Read the model definition and answer for the solid it produces. Units are mm, in the model's axes. A direction names the side the tool comes from. Give positions to 0.01 mm unless a question says otherwise; leave off trailing zeros. Order: outer loops, then holes, each group sorted by start corner. A loop starts at its lowest first (then second) coordinate and runs counter-clockwise, first axis right, second up. Notation, with made-up numbers: M 23,86 L 42,86 A25 ccw 42,123 Z; hole C 61,73.25 d2. An arc over 180 degrees is marked long. One line per item, written item: value.
from build123d import *
from OCP.BRepFilletAPI import BRepFilletAPI_MakeChamfer

# Parameters (mm, degrees)
SKETCH2_R           = 110
BOSS_EXTRUDE1_DEPTH = 26
CUT_EXTRUDE1_DEPTH  = 26
CHAMFER1_SIZE       = 2
CHAMFER2_SIZE       = 10
CHAMFER2_SIZE2      = 5.773502692
SKETCH4_R           = 85
CUT_EXTRUDE2_DEPTH  = 26
CHAMFER3_SIZE       = 2


with BuildPart() as part:
    # Sketch2 → Boss-Extrude1 (new body)
    with BuildSketch(Plane.XY):
        with Locations(Location((0, 0, 0), (0, 0, 180))):
            Circle(SKETCH2_R)
    extrude(amount=BOSS_EXTRUDE1_DEPTH)

    # Sketch3 → Cut-Extrude1 (cut)
    with BuildSketch(Plane.XY.offset(26)):
        with BuildLine():
            Line((-8, 109.954040528), (-8, 103))
            Line((-8, 103), (8, 103))
            Line((8, 103), (8, 109.954040528))
            ThreePointArc((8, 109.954040528), (0, 110.244687076), (-8, 109.954040528))
        make_face()
        with BuildLine():
            Line((-109.954040528, -8), (-103, -8))
            Line((-103, -8), (-103, 8))
            Line((-103, 8), (-109.954040528, 8))
            ThreePointArc((-109.954040528, 8), (-110.244687076, 0), (-109.954040528, -8))
        make_face()
        with BuildLine():
            Line((103, 8), (103, -8))
            Line((103, -8), (109.954040528, -8))
            ThreePointArc((109.954040528, -8), (110.244687076, 0), (109.954040528, 8))
            Line((109.954040528, 8), (103, 8))
        make_face()
        with BuildLine():
            Line((-8, -103), (-8, -109.954040528))
            ThreePointArc((-8, -109.954040528), (0, -110.244687076), (8, -109.954040528))
            Line((8, -109.954040528), (8, -103))
            Line((8, -103), (-8, -103))
        make_face()
    extrude(amount=-CUT_EXTRUDE1_DEPTH, mode=Mode.SUBTRACT)

    # Chamfer1
    chamfer1_edges = [part.edges().sort_by_distance(p)[0] for p in [
        (-77.781745931, 77.781745931, 26),
        (77.781745931, 77.781745931, 26),
        (-77.781745931, -77.781745931, 26),
        (77.781745931, -77.781745931, 26),
    ]]
    chamfer(chamfer1_edges, length=CHAMFER1_SIZE)

    # Chamfer2: one chamfer whose edges measure the first distance from different faces: ONE call of the kernel's chamfer builder (chamfer() names one face for all edges)
    chamfer2_edges_1 = [part.edges().sort_by_distance(p)[0] for p in [
        (77.781745931, 77.781745931, 0),
    ]]
    chamfer2_side_1 = [part.faces().sort_by_distance(p)[0] for p in [
        (77.781745931, 77.781745931, 12),
    ]]
    chamfer2_edges_2 = [part.edges().sort_by_distance(p)[0] for p in [
        (-77.781745931, 77.781745931, 0),
    ]]
    chamfer2_side_2 = [part.faces().sort_by_distance(p)[0] for p in [
        (-77.781745931, 77.781745931, 12),
    ]]
    chamfer2_edges_3 = [part.edges().sort_by_distance(p)[0] for p in [
        (-77.781745931, -77.781745931, 0),
    ]]
    chamfer2_side_3 = [part.faces().sort_by_distance(p)[0] for p in [
        (-77.781745931, -77.781745931, 12),
    ]]
    chamfer2_edges_4 = [part.edges().sort_by_distance(p)[0] for p in [
        (77.781745931, -77.781745931, 0),
    ]]
    chamfer2_side_4 = [part.faces().sort_by_distance(p)[0] for p in [
        (77.781745931, -77.781745931, 12),
    ]]
    chamfer2 = BRepFilletAPI_MakeChamfer(part.part.solid().wrapped)
    for e in chamfer2_edges_1:
        chamfer2.Add(CHAMFER2_SIZE, CHAMFER2_SIZE2, e.wrapped, chamfer2_side_1[0].wrapped)  # the first distance lies on this face
    for e in chamfer2_edges_2:
        chamfer2.Add(CHAMFER2_SIZE, CHAMFER2_SIZE2, e.wrapped, chamfer2_side_2[0].wrapped)  # the first distance lies on this face
    for e in chamfer2_edges_3:
        chamfer2.Add(CHAMFER2_SIZE, CHAMFER2_SIZE2, e.wrapped, chamfer2_side_3[0].wrapped)  # the first distance lies on this face
    for e in chamfer2_edges_4:
        chamfer2.Add(CHAMFER2_SIZE, CHAMFER2_SIZE2, e.wrapped, chamfer2_side_4[0].wrapped)  # the first distance lies on this face
    add(Compound.cast(chamfer2.Shape()), mode=Mode.REPLACE)

    # Sketch4 → Cut-Extrude2 (cut)
    with BuildSketch(Plane(origin=(0, 0, 0), x_dir=(-1, 0, 0), z_dir=(0, 0, -1))):
        Circle(SKETCH4_R)
    extrude(amount=-CUT_EXTRUDE2_DEPTH, mode=Mode.SUBTRACT)

    # Chamfer3
    chamfer3_edges = [part.edges().sort_by_distance(p)[0] for p in [
        (85, 0, 26),
        (85, 0, 0),
    ]]
    chamfer(chamfer3_edges, length=CHAMFER3_SIZE)


solid = part.part
1) Which of the six approach directions +Z, -Z, +X, -X, +Y, -Y give full straight-line access (tool end or side, diameter ignored) to faces 4 (the face through (8, 106, 16)), 5 (the face through (-79, 39, 26)), 6 (the face through (0, -103, 13)), 7 (the face through (-75.1, -73.6, 1.6)), 8 (the face through (-103, 0, 13))?
Reported:
face 4: +Z, -Z, +Y
face 5: +Z, +X, -X, +Y, -Y
face 6: +Z, -Z, -Y
face 7: -Z, -X, -Y
face 8: +Z, -Z, -X
2) Find section A-A, the plane x = 0. Write down the section's boundary in (y, z).
Reported:
outline: M -103,0 L -87,0 L -85,2 L -85,24 L -87,26 L -103,26 Z; M 85,2 L 87,0 L 103,0 L 103,26 L 87,26 L 85,24 Z
3) Each of these flat-tipped pins is pushed along its axis until it touches: pin 1 Ø1 at (y, z) = (-69, 7.5) entering from +X; pin 2 Ø13 at (y, z) = (-2.5, 11.5) entering from +X; pin 3 Ø8 at (y, z) = (79, 5.5) entering from +X; pin 4 Ø1.5 at (x, z) = (83.5, 9.5) entering from +Y. Where does it stop, or does it pass through?
Reported:
pin 1: stops at x = 84.36
pin 2: stops at x = 109.71
pin 3: stops at x = 78.04
pin 4: stops at y = 72.26
4) Consider probe 1 along Y at (x, z) = (0, 16.25); probe 2 along Y at (x, z) = (63, 16); probe 3 along X at (y, z) = (-40.5, 7.75). Determine where each line is inside the solid, lowest interval first.
Reported:
probe 1: y = -103 to -85, 85 to 103
probe 2: y = -90.17 to -57.06, 57.06 to 90.17
probe 3: x = -100.87 to -74.73, 74.73 to 100.87
5) Find section C-C, the plane z = 14.5. Write down the section's boundary in (x, y), plus the area to 3 significant figures.
Reported:
outline: M -109.71,-8 A110 ccw -8,-109.71 L -8,-103 L 8,-103 L 8,-109.71 A110 ccw 109.71,-8 L 103,-8 L 103,8 L 109.71,8 A110 ccw 8,109.71 L 8,103 L -8,103 L -8,109.71 A110 ccw -109.71,8 L -103,8 L -103,-8 Z; hole C 0,0 d170
area: 14,900 mm^2
6) Determine the mould class of faces 1 (the face through (-106, 8, 16)), 2 (the face through (-78.554, -77.002, 16.902)), 3 (the face through (8, -106, 16)) for opening direction X: +X half, -X half, draft (parallel to the pull), parting line (faces both ways), or undercut.
Reported:
face 1: draft
face 2: -X half
face 3: undercut
